Could you check a few things on this drawing? It's one solid part, dimensions in mm from its lowest x, y, z. A direction names the side the tool comes from. Round coordinates to 2 decimals unless told otherwise and drop trailing zeros. Loops run counter-clockwise (first coordinate to the right, second up) from the corner with the lowest first, then second, coordinate; pieces in that order, holes last. Notation, with made-up numbers: M 76,5.5 L 85,5.5 A19 cw 85,41.5 Z; hole C 13,-31.75 d3. An arc over 180 degrees is marked long. Return JSON: item names as keys, results as strings.
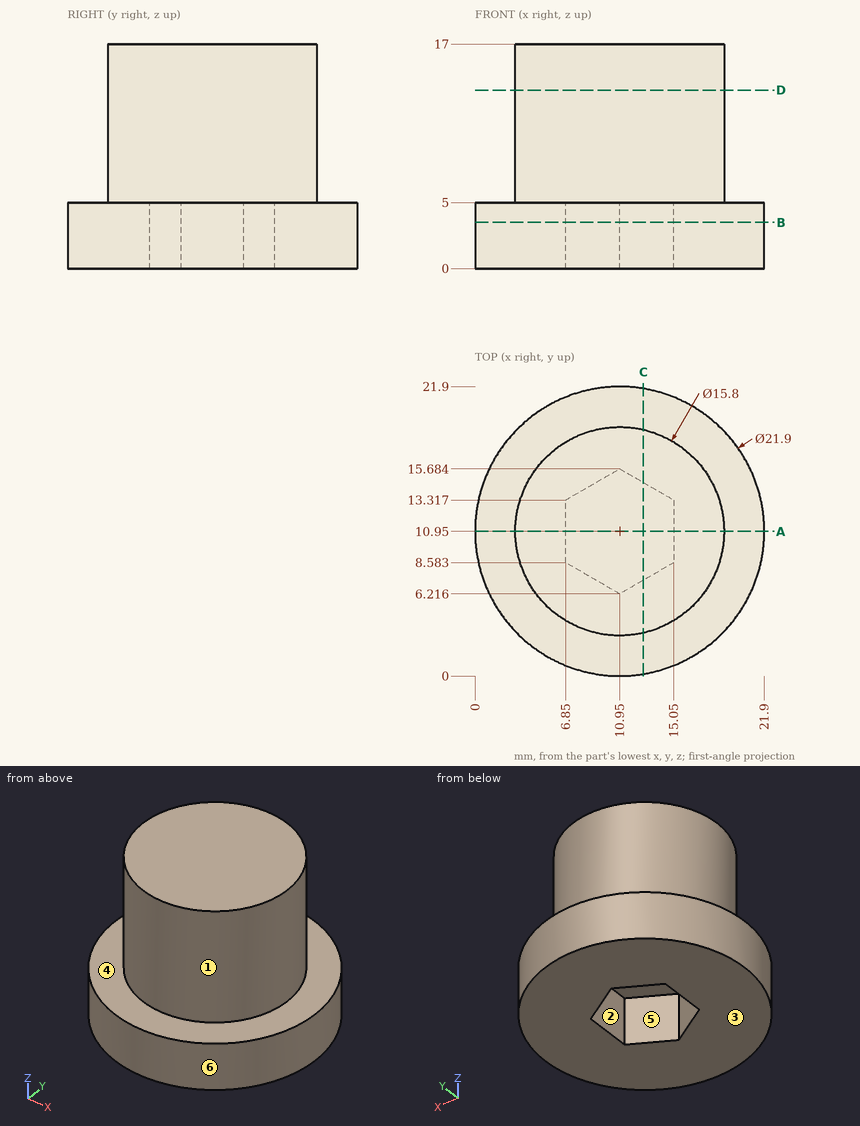
Q1. If I drill on line 1 along Z through (x, y) = (6.75, 17.75); line 2 along X through (y, z) = (14.5, 4.5); line 3 along Y through (x, z) = (13.75, 4.75) (1 decimal), over which ranges is the centre line in solid material (lowest first)?
Results:
{"line 1": "z = 0 to 5", "line 2": "x = 0.59 to 8.9, 13 to 21.31", "line 3": "y = 0.4 to 7.8, 14.1 to 21.5"}
Q2. I'm going to push flat-ended pins straight in: pin 1 Ø3 at (y, z) = (15, 4) entering from +X; pin 2 Ø1.5 at (y, z) = (6.5, 13) entering from +X; pin 3 Ø8 at (y, z) = (6, 8.5) entering from -X. Where does each tip first touch, or does it pass through?
Results:
{"pin 1": "stops at x = 21.6", "pin 2": "stops at x = 17.93", "pin 3": "stops at x = 0.42"}
Q3. Thinking about a two-plate mould opening in Y: for the marked faces 1, 2 and 3, which applies, pulls with the +Y half, pulls with the -Y half, needs draft (parallel to the pull), parting line crosses it, or undercut?
Results:
{"face 1": "parting line crosses it", "face 2": "undercut", "face 3": "needs draft"}
Q4. Suppose I cut it at C-C, the plane x = 12.75. Please give me the cut outline in (y, z) (1 decimal).
Results:
{"outline": "M 0.1,0 L 7.3,0 L 7.3,5 L 14.6,5 L 14.6,0 L 21.8,0 L 21.8,5 L 18.6,5 L 18.6,17 L 3.3,17 L 3.3,5 L 0.1,5 Z"}
Q5. Suppose I cut it at A-A, the plane y = 10.95. Please give me the cut outline in (x, z).
Results:
{"outline": "M 0,0 L 6.85,0 L 6.85,5 L 15.05,5 L 15.05,0 L 21.9,0 L 21.9,5 L 18.85,5 L 18.85,17 L 3.05,17 L 3.05,5 L 0,5 Z"}
Q6. On a 3-axis mill with a long thin cutter (end or side, diameter ignored), from which of +Z, -Z, +X, -X, +Y, -Y can I reach the whole of each face in a straight line? I mean the marked faces 4, 5 and 6. Say none if no direction works.
Results:
{"face 4": "+Z", "face 5": "-Z", "face 6": "+Z, -Z"}
Q7. Suppose I cut it at B-B, the plane z = 3.5. Please give me the cut outline in (x, y).
Results:
{"outline": "C 10.95,10.95 d21.9; hole M 6.85,8.58 L 10.95,6.22 L 15.05,8.58 L 15.05,13.32 L 10.95,15.68 L 6.85,13.32 Z"}
Q8. Suppose I cut it at D-D, the plane z = 13.5. Please give me the cut outline in (x, y), plus the area to 3 significant figures.
Results:
{"outline": "C 10.95,10.95 d15.8", "area": "196 mm2"}
